Verification items for this drawing (mm, ordinates from the low corner). A direction names the side the tool comes from. Give positions to 0.01 mm unless a question says otherwise; leave off trailing zeros. Loops run counter-clockwise (first coordinate to the right, second up) from the corner with the lowest first, then second, coordinate; pieces in that order, holes last. Notation, with made-up numbers: (-19, 31) - (5, 31) arc R23 cw to (5, 49) - close; hole circle Ø7 at (-29.5, 69). An arc over 180 degrees is marked (long way). One line per question, with ' | ' between items. Start each with the question number.
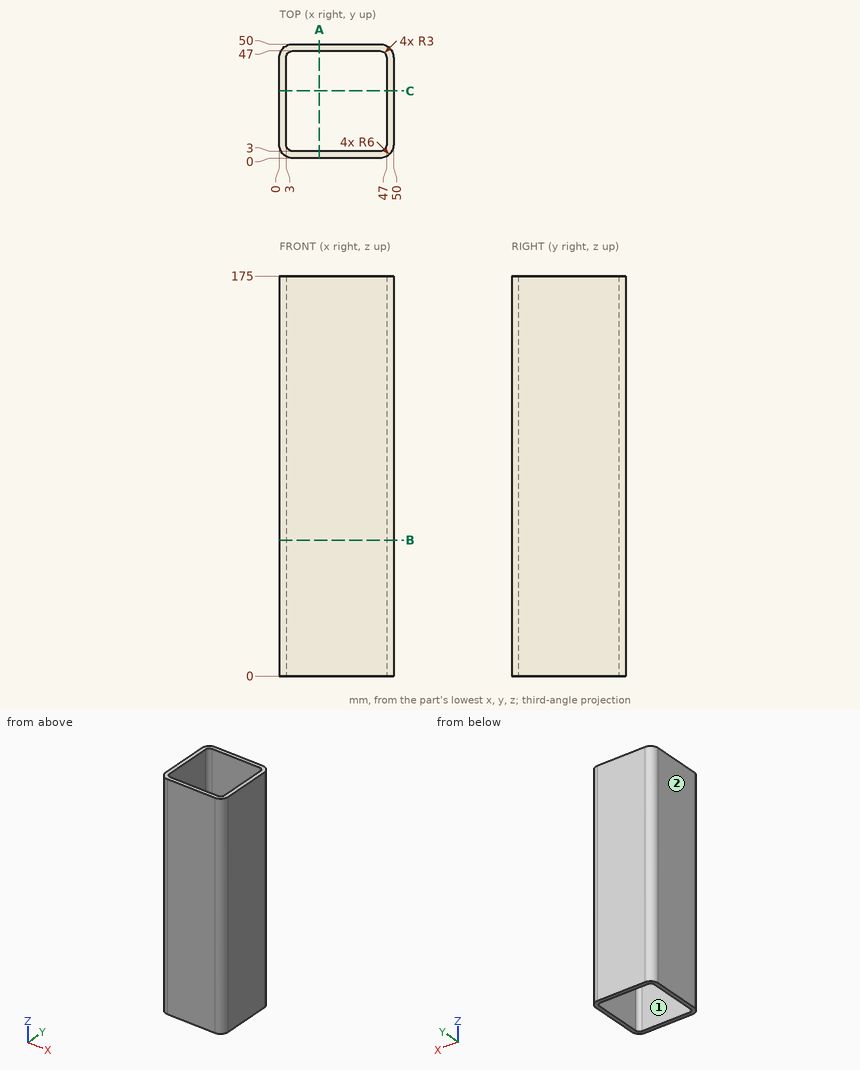
(1) Tool access check on the marked faces 1 and 2. Record the directions out of +Z, -Z, +X, -X, +Y, -Y that give a thin tool (end or side, any length) a straight path to the whole face; none if there is none.
(2) Section check A-A, the plane x = 17.5. Record the boundary of the cut face in (y, z), and give its area (3 significant figures).
(3) Material ranges on line 1 (Y direction, x = 44, z = 8); line 2 (X direction, y = 4, z = 150), recorded low to high.
(4) Section check B-B, the plane z = 59.5. Record the boundary of the cut face in (x, y).
Numbers:
1) face 1: +Z, -Z | face 2: +Z, -Z, -X, +Y, -Y
2) outline: (0, 0) - (3, 0) - (3, 175) - (0, 175) - close; (47, 0) - (50, 0) - (50, 175) - (47, 175) - close | area: 1,050 mm^2
3) line 1: 0 to 3, 47 to 50 | line 2: 0.34 to 3.76, 46.24 to 49.66
4) outline: (0, 6) arc R6 ccw to (6, 0) - (44, 0) arc R6 ccw to (50, 6) - (50, 44) arc R6 ccw to (44, 50) - (6, 50) arc R6 ccw to (0, 44) - close; hole (3, 6) arc R3 ccw to (6, 3) - (44, 3) arc R3 ccw to (47, 6) - (47, 44) arc R3 ccw to (44, 47) - (6, 47) arc R3 ccw to (3, 44) - close
